Design review of the part shown in the three views and the two pictorial views. Dimensions are in mm from the part's minimum x, y and z. A direction names the side the tool comes from. Coordinates: 2 decimals unless noted, no trailing zeros. Order: outer loops, then holes, each group sorted by start corner. A loop starts at its lowest first (then second) coordinate and runs counter-clockwise, first axis right, second up. Notation, with made-up numbers: (71, -17) -> (113, -17) arc R30 cw to (113, 13) -> close; hole circle Ø3 at (71.5, -35.75). An arc over 180 degrees is marked (long way). Write item = value, one per line. Start each with the question number.
1) Consider section A-A on x = 183. Give the boundary of the cut face in (y, z).
2) Consider section B-B on x = 121. Give the boundary of the cut face in (y, z) (1 decimal).
3) Consider section D-D on y = 43.5. Give the boundary of the cut face in (x, z).
4) Machinability: for the marked faces 5, 6, 7 and 8, which of the approach directions +Z, -Z, +X, -X, +Y, -Y give a long, thin tool a straight path to every point of the face, cutting with its end or side? Answer none if there is none.
5) Consider section C-C on x = 148. Give the boundary of the cut face in (y, z).
6) Wall thickness on probe 1 along Y at (x, z) = (179, 53); probe 2 along X at (y, z) = (11.5, 80); probe 3 along X at (y, z) = (12, 136): over which ranges is each line inside the solid? List them lowest first. Write a range as [from, to].
7) Insertion check: pin 1 Ø22 at (x, y) = (162, 89) entering from +Z; pin 2 Ø22 at (x, y) = (42.5, 86.5) entering from +Z; pin 3 Ø5 at (x, y) = (134.5, 20.5) entering from +Z. Each pin has a flat end and moves straight along its axis. Give the tip position at first contact, or say it passes through.
8) Draft analysis for pull direction X (two halves, no side actions). For the marked faces 1, 2, 3 and 4, state which applies: +X half, -X half, draft (parallel to the pull), parting line (faces both ways), or undercut.
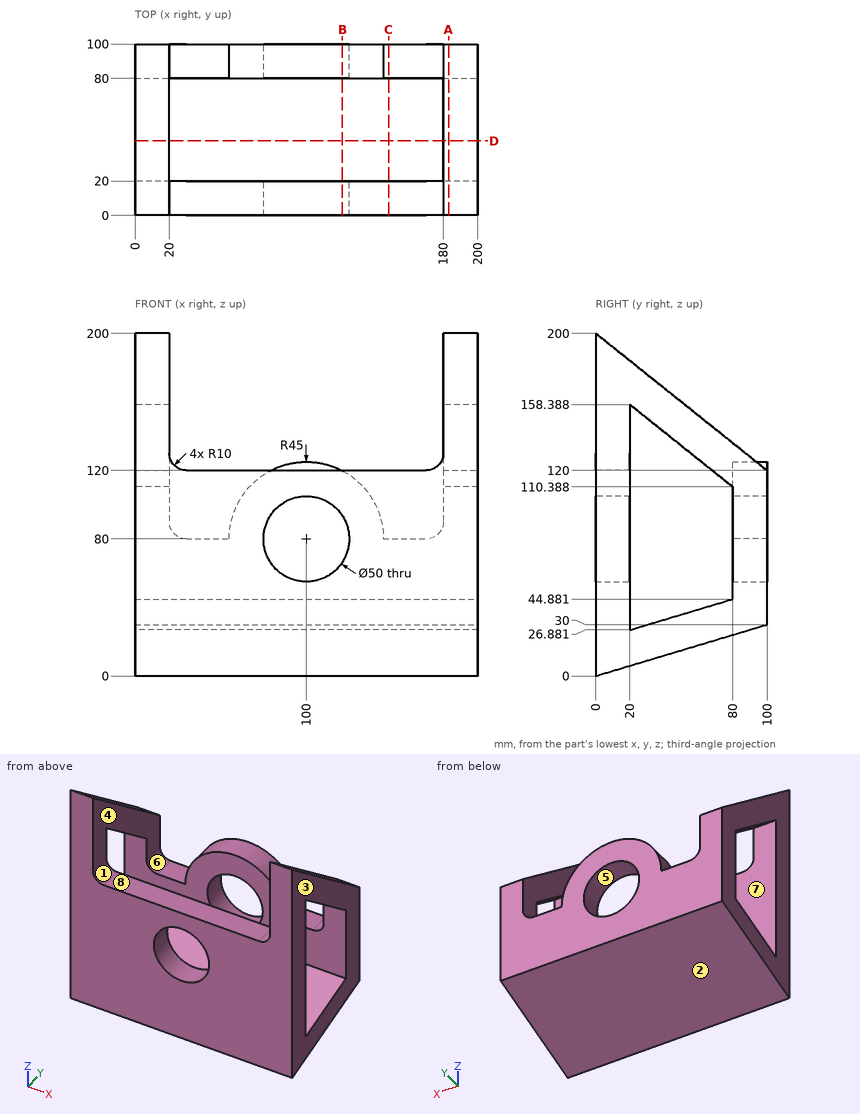
Answer sheet:
q1.outline = (0, 0) -> (100, 30) -> (100, 120) -> (0, 200) -> close; hole (20, 26.88) -> (80, 44.88) -> (80, 110.39) -> (20, 158.39) -> close
q2.outline = (0, 0) -> (100, 30) -> (100, 66.4) -> (80, 66.4) -> (80, 44.9) -> (20, 26.9) -> (20, 66.4) -> (0, 66.4) -> close; (0, 93.6) -> (20, 93.6) -> (20, 120) -> (0, 120) -> close; (80, 93.6) -> (100, 93.6) -> (100, 119.8) -> (80, 119.8) -> close
q3.outline = (0, 13.05) -> (200, 13.05) -> (200, 33.93) -> (0, 33.93) -> close; (0, 139.59) -> (20, 139.59) -> (20, 165.2) -> (0, 165.2) -> close; (180, 139.59) -> (200, 139.59) -> (200, 165.2) -> (180, 165.2) -> close
q4.face_5 = +Y, -Y
q4.face_6 = +Z, +Y
q4.face_7 = +X, -X
q4.face_8 = +Z, -Y
q5.outline = (0, 0) -> (100, 30) -> (100, 80) -> (80, 80) -> (80, 44.88) -> (20, 26.88) -> (20, 120) -> (0, 120) -> close
q6.probe_1 = [0, 20], [80, 100]
q6.probe_2 = [0, 75], [125, 200]
q6.probe_3 = [0, 20], [180, 200]
q7.pin_1 = 80.46
q7.pin_2 = 80
q7.pin_3 = 120
q8.face_1 = undercut
q8.face_2 = draft
q8.face_3 = +X half
q8.face_4 = undercut
